```python
from build123d import *

# Parameters (mm, degrees)
SECTION_SIZE_W                              = 35
SECTION_SIZE_H                              = 23.5
SECTION_SIZE_W_2                            = 25
SECTION_SIZE_H_2                            = 18
SKETCH2_W                                   = 35
SKETCH2_H                                   = 30
FITTING114_4_12PZ_1_DEPTH                   = 2.75
SKETCH6_W                                   = 35
SKETCH6_H                                   = 30
FITTING114_4_12PZ_2_DEPTH                   = 2.75
RIB_E_REACH                                 = 379.167
SKETCH9_WALL_W                              = 783.159137046
SKETCH9_WALL_H                              = 4.1
RIB_Z_REACH                                 = 379.167
SKETCH10_WALL_W                             = 783.159137046
SKETCH10_WALL_H                             = 4.1
M5_FLAT_HEAD_SCREW_COUNTERSINK1_AT_2_COUNT  = 2
M5_FLAT_HEAD_SCREW_COUNTERSINK1_AT_2_PITCH  = 13.862178761
M5_FLAT_HEAD_SCREW_COUNTERSINK1_AT_3_COUNT  = 2
M5_FLAT_HEAD_SCREW_COUNTERSINK1_AT_3_PITCH  = 19.2
M5_FLAT_HEAD_SCREW_COUNTERSINK2_D           = 5.5
M5_FLAT_HEAD_SCREW_COUNTERSINK2_DEPTH       = 35
M5_FLAT_HEAD_SCREW_COUNTERSINK2_CSINK_D     = 10.4
M5_FLAT_HEAD_SCREW_COUNTERSINK2_CSINK_ANGLE = 90
M5_FLAT_HEAD_SCREW_COUNTERSINK2_TIP         = 1.652366702


with BuildPart() as part:
    # Chain: sweep along a path in Length Path
    with BuildLine(Plane(origin=(0, 0, 0), x_dir=(0, 0, -1), z_dir=(1, 0, 0))) as chain_path:
        Line((-250, 96), (-300, 96))
        ThreePointArc((-300, 96), (-348, 48), (-300, 0))
        Line((-300, 0), (0, 0))
    # Section Size → Chain (sweep)
    with BuildSketch(Plane.XY):
        Rectangle(SECTION_SIZE_W, SECTION_SIZE_H)
        Rectangle(SECTION_SIZE_W_2, SECTION_SIZE_H_2, mode=Mode.SUBTRACT)
    sweep(path=chain_path.line)

    # Sketch2 → Fitting114.4.12PZ-1 (add)
    with BuildSketch(Plane(origin=(0, 84.25, 0), x_dir=(1, 0, 0), z_dir=(0, 1, 0))):
        with Locations((0, -235)):
            Rectangle(SKETCH2_W, SKETCH2_H)
    extrude(amount=FITTING114_4_12PZ_1_DEPTH)

    # Sketch6 → Fitting114.4.12PZ-2 (add)
    with BuildSketch(Plane.XZ.offset(11.75)):
        with Locations((0, -15)):
            Rectangle(SKETCH6_W, SKETCH6_H)
    extrude(amount=-FITTING114_4_12PZ_2_DEPTH)

    # Sketch9 wall → E (add, up to next)
    with BuildSketch(Plane(origin=(17.5, 97.375, 241.5), x_dir=(0, -0.773541895, -0.633745166988), z_dir=(0, 0.633745166988, -0.773541895)), mode=Mode.PRIVATE) as rib_e_sk1:
        with Locations((0, 2.05)):
            Rectangle(SKETCH9_WALL_W, SKETCH9_WALL_H)
    rib_e_tool1 = extrude(rib_e_sk1.sketch, amount=-RIB_E_REACH, mode=Mode.PRIVATE) - part.part
    rib_e = rib_e_tool1.solids().sort_by_distance((17.5, 97.375, 241.5))[0]
    add(rib_e)

    # Sketch10 wall → Z (add, up to next)
    with BuildSketch(Plane(origin=(17.5, 1.375, -8.5), x_dir=(0, 0.773541895, 0.633745166988), z_dir=(0, -0.633745166988, 0.773541895)), mode=Mode.PRIVATE) as rib_z_sk1:
        with Locations((0, 2.05)):
            Rectangle(SKETCH10_WALL_W, SKETCH10_WALL_H)
    rib_z_tool1 = extrude(rib_z_sk1.sketch, amount=RIB_Z_REACH, mode=Mode.PRIVATE) - part.part
    rib_z = rib_z_tool1.solids().sort_by_distance((17.5, 1.375, -8.5))[0]
    add(rib_z)

    # Drag: E, Z across plane
    add(rib_e.mirror(Plane(origin=(0, 0, 0), x_dir=(0, 0, 1), z_dir=(1, 0, 0))))
    add(rib_z.mirror(Plane(origin=(0, 0, 0), x_dir=(0, 0, 1), z_dir=(1, 0, 0))))

    # Sketch17 → M5 Flat Head Screw Countersink1 (revolve, cut)
    with BuildSketch(Plane(origin=(-9.6, -9, -23), x_dir=(0, 0, 1), z_dir=(1, 0, 0))):
        Polygon((0, 0), (0, 2.75), (2.75, 2.75), (2.75, 2.45), (5.2, 0), align=None)
    m5_flat_head_screw_countersink1 = revolve(axis=Axis((-9.6, -2.65, -23), (0, -1, 0)), mode=Mode.SUBTRACT)

    # M5 Flat Head Screw Countersink1 at 2: M5 Flat Head Screw Countersink1 ×2
    with Locations(*[Vector(0.6925318281897137, 0, 0.7213873210309515) * (i * M5_FLAT_HEAD_SCREW_COUNTERSINK1_AT_2_PITCH) for i in range(1, M5_FLAT_HEAD_SCREW_COUNTERSINK1_AT_2_COUNT)]):
        add(m5_flat_head_screw_countersink1, mode=Mode.SUBTRACT)

    # M5 Flat Head Screw Countersink1 at 3: M5 Flat Head Screw Countersink1 ×2
    with Locations(*[(i * M5_FLAT_HEAD_SCREW_COUNTERSINK1_AT_3_PITCH, 0, 0) for i in range(1, M5_FLAT_HEAD_SCREW_COUNTERSINK1_AT_3_COUNT)]):
        add(m5_flat_head_screw_countersink1, mode=Mode.SUBTRACT)

    # M5 Flat Head Screw Countersink2
    with Locations(Plane(origin=(-9.6, 87, 227), x_dir=(0, 0, 1), z_dir=(0, 1, 0))):
        with Locations((0, 0), (10, 9.6), (0, 19.2)):
            CounterSinkHole(M5_FLAT_HEAD_SCREW_COUNTERSINK2_D / 2, M5_FLAT_HEAD_SCREW_COUNTERSINK2_CSINK_D / 2, depth=M5_FLAT_HEAD_SCREW_COUNTERSINK2_DEPTH, counter_sink_angle=M5_FLAT_HEAD_SCREW_COUNTERSINK2_CSINK_ANGLE)
            with Locations((0, 0, -(M5_FLAT_HEAD_SCREW_COUNTERSINK2_DEPTH + M5_FLAT_HEAD_SCREW_COUNTERSINK2_TIP / 2))):  # 118° drill point
                Cone(0, M5_FLAT_HEAD_SCREW_COUNTERSINK2_D / 2, M5_FLAT_HEAD_SCREW_COUNTERSINK2_TIP, mode=Mode.SUBTRACT)


solid = part.part
```
Can you work these out from the model? Positions are in its coordinate system, mm. A direction names the side the tool comes from. Give positions to 0.01 mm unless a question says otherwise; leave off trailing zeros. Loops run counter-clockwise (first coordinate to the right, second up) from the corner with the lowest first, then second, coordinate; pieces in that order, holes last. Notation, with made-up numbers: M -27.5,-40 L 17.5,-40 A33 ccw 17.5,-10 Z; hole C -13.5,33.25 d2. An arc over 180 degrees is marked long. Use one line per item in the form item = value. Start each with the question number.
(1) On a 3-axis mill with a long thin cutter (end or side, diameter ignored), from which of +Z, -Z, +X, -X, +Y, -Y can I reach the whole of each face in a straight line? I mean faces 1 (the cylindrical face through (0.18, 48.86, 338.99)), 2 (the flat face through (-13.4, 95, 244)), 3 (the flat face through (0, 84.25, 259)), 4 (the flat face through (-17.5, 6, 215)). Say none if no direction works.
(2) I want a section at A-A, the plane z = 33.5. Write out the boundary of the cut face in (x, y).
(3) I want a section at B-B, the plane y = 48. Write out the boundary of the cut face in (x, z).
(4) Please list where these lines run through material, in increasing order: line 1 (Y direction, x = 0, z = 279); line 2 (X direction, y = -11.7, z = -23); line 3 (X direction, y = -11.55, z = -13).
(5) Thinking about a two-plate mould opening in Y: for faces 5 (the cylindrical face through (-0.175, 49.253, 356.986)), 6 (the flat face through (1, 106, 250)), 7 (the conical face through (9.7, 84.7, 229.9)), which applies, released by +Y, released by -Y, zero draft, split by the parting line, or undercut?
(6) I'm going to push flat-ended pins straight in: P1, Ø6, axis at x = 8.5, z = 65, coming from the +Y side; P2, Ø3, axis at x = -12.5, y = 61.5, coming from the -Z side; P3, Ø5, axis at x = -12.5, y = 36.5, coming from the -Z side. Where does each tip first touch, or does it pass through?
(7) I want a section at C-C, the plane y = -1. Write out the boundary of the cut face in (x, z), and give its area (3 significant figures).
Worked out:
q1.face_1 = none
q1.face_2 = -Z, +Y
q1.face_3 = -Z, +X, -X
q1.face_4 = +Z, -Z, -X, +Y, -Y
q2.outline = M -17.5,-11.75 L 17.5,-11.75 L 17.5,11.75 L -17.5,11.75 Z; hole M -12.5,-9 L 12.5,-9 L 12.5,9 L -12.5,9 Z
q3.outline = M -17.5,336.25 L 17.5,336.25 L 17.5,359.75 L -17.5,359.75 Z; hole M -12.5,339 L 12.5,339 L 12.5,357 L -12.5,357 Z
q4.line_1 = -11.75 to -9, 9 to 11.75, 84.25 to 87, 105 to 107.75
q4.line_2 = -17.5 to -12.35, -6.85 to 6.85, 12.35 to 17.5
q4.line_3 = -17.5 to -2.75, 2.75 to 17.5
q5.face_5 = undercut
q5.face_6 = zero draft
q5.face_7 = released by +Y
q6.P1 = 11.75
q6.P2 = 333
q6.P3 = 333.44
q7.outline = M -17.5,-10.45 L -13.4,-10.45 L -13.4,0 L -12.5,0 L -12.5,329.12 L 12.5,329.12 L 12.5,0 L 13.4,0 L 13.4,-10.45 L 17.5,-10.45 L 17.5,334.19 L -17.5,334.19 Z
q7.area = 3,550 mm²
